Geometry check sheet. Reference: drawing and pictorial views, mm from the part's lowest x, y, z. A direction names the side the tool comes from. Give positions to 0.01 mm unless a question says otherwise; leave off trailing zeros. Write each loop counter-clockwise with the first axis right and the second up, starting at its lowest first coordinate (ties: lowest second). Pieces come first, ordered by that corner, then holes. Notation, with made-up numbers: M 86,67 L 92,67 A25 ccw 92,98 Z; hole C 84,-19 d5. An arc over 180 degrees is marked long. Answer as a JSON object with one key per item and string values.
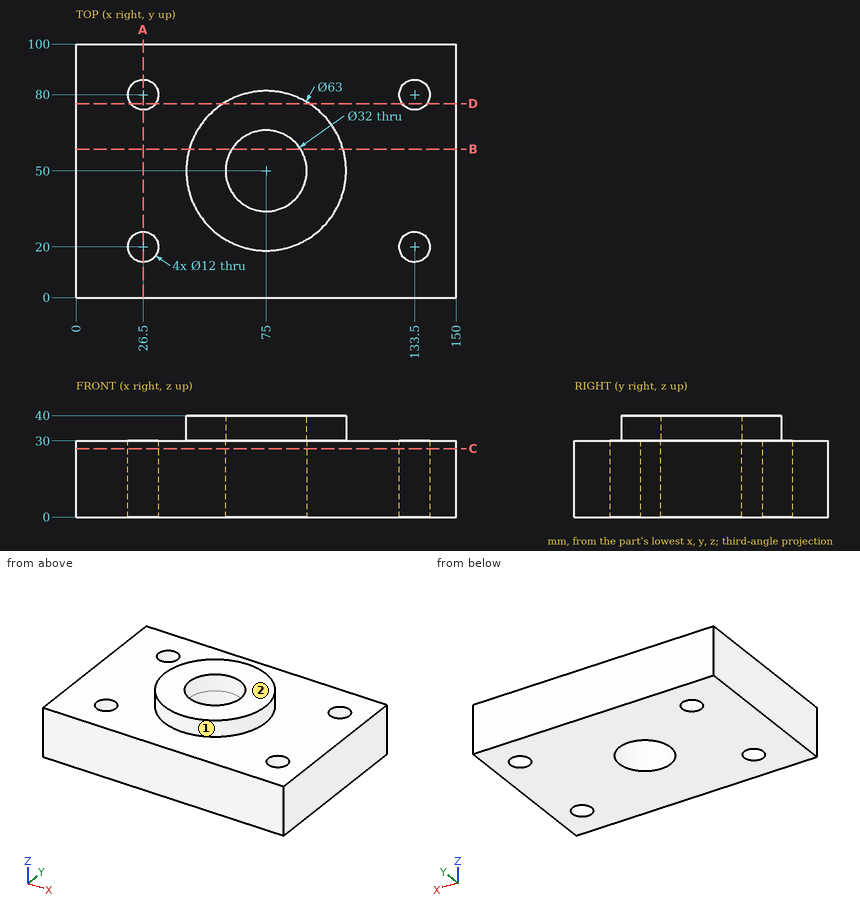
1) Section check C-C on z = 27. Record the boundary of the cut face in (x, y), and give its area (3 significant figures).
Completed:
{"outline": "M 0,0 L 150,0 L 150,100 L 0,100 Z; hole C 26.5,20 d12; hole C 26.5,80 d12; hole C 75,50 d32; hole C 133.5,20 d12; hole C 133.5,80 d12", "area": "13,700 mm2"}
2) Section check B-B on y = 58.5. Record the boundary of the cut face in (x, z), and give its area (3 significant figures).
Completed:
{"outline": "M 0,0 L 61.44,0 L 61.44,40 L 44.67,40 L 44.67,30 L 0,30 Z; M 88.56,0 L 150,0 L 150,30 L 105.33,30 L 105.33,40 L 88.56,40 Z", "area": "4,020 mm2"}
3) Section check A-A on x = 26.5. Record the boundary of the cut face in (y, z), and give its area (3 significant figures).
Completed:
{"outline": "M 0,0 L 14,0 L 14,30 L 0,30 Z; M 26,0 L 74,0 L 74,30 L 26,30 Z; M 86,0 L 100,0 L 100,30 L 86,30 Z", "area": "2,280 mm2"}
4) Thickness scan on L1, parallel to Y at x = 133, z = 10; L2, parallel to X at y = 44, z = 17.5; L3, parallel to Y at x = 86, z = 3.5. Record the ranges inside material, lowest first.
Completed:
{"L1": "y = 0 to 14.02, 25.98 to 74.02, 85.98 to 100", "L2": "x = 0 to 60.17, 89.83 to 150", "L3": "y = 0 to 38.38, 61.62 to 100"}
5) Access from +Z, -Z, +X, -X, +Y, -Y to the whole of each face (thin tool, end or side, straight path). Record for the marked faces 1 and 2.
Completed:
{"face 1": "+Z", "face 2": "+Z, +X, -X, +Y, -Y"}
6) Section check D-D on y = 76.5. Record the boundary of the cut face in (x, z), and give its area (3 significant figures).
Completed:
{"outline": "M 0,0 L 21.63,0 L 21.63,30 L 0,30 Z; M 31.37,0 L 128.63,0 L 128.63,30 L 92.03,30 L 92.03,40 L 57.97,40 L 57.97,30 L 31.37,30 Z; M 138.37,0 L 150,0 L 150,30 L 138.37,30 Z", "area": "4,260 mm2"}
